Study the drawing (mm; zero at the part's minimum x, y, z) and answer. A direction names the side the tool comes from. Coordinates: 2 decimals unless noted, no trailing zeros. Order: outer loops, then holes, each group sorted by start corner. A loop starts at its lowest first (then second) coordinate and runs counter-clockwise, first axis right, second up.
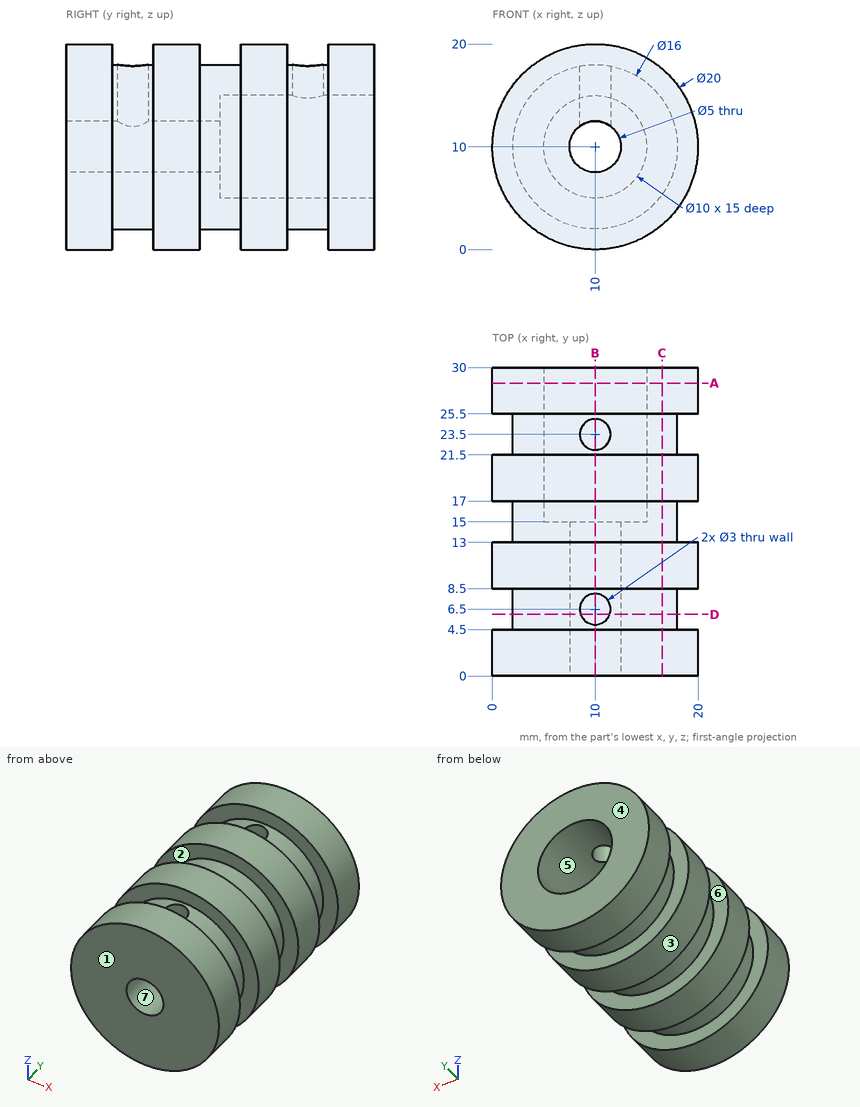
(1) Find section B-B on x = 10. Count the separate pieces of the cut face and the enclosed holes in it, then the cut area to 4 significant figures.
(2) Find section A-A on y = 28.5. Determine the outline of the cut face in (x, z).
(3) The mould has two halves that part along Y. Classify the marked faces 1, 2, 3 and 4: pulls with the +Y half, pulls with the -Y half, needs draft (parallel to the pull), parting line crosses it, or undercut.
(4) Given pin 1 Ø2 at (x, y) = (3, 17.5) entering from +Z; pin 2 Ø12 at (y, z) = (8, 17) entering from +X; pin 3 Ø1.5 at (x, y) = (11, 21) entering from +Z, each flat-ended and moving along its own axis, determine where each tip first touches the part or whether it passes through.
(5) Find section D-D on y = 6. Determine the outline of the cut face in (x, z).
(6) A tool of negligible diameter and unlimited length cuts with its end or side. For the marked faces 5, 6 and 7, from which of +Z, -Z, +X, -X, +Y, -Y can it reach the whole face along a straight path? Write none if from no direction.
(7) Find section C-C on x = 16.5. Determine the outline of the cut face in (y, z).
(8) Find the intervals of material crossed by probe 1 along Y at (x, z) = (14.75, 2.5); probe 2 along Y at (x, z) = (10, 15.5); probe 3 along X at (y, z) = (4.25, 10), in increasing order.
Resolved:
1. separate pieces: 4
1. enclosed holes: 0
1. area: 301.5 mm2
2. outline: circle Ø20 at (10, 10); hole circle Ø10 at (10, 10)
3. face 1: pulls with the -Y half
3. face 2: undercut
3. face 3: needs draft
3. face 4: pulls with the +Y half
4. pin 1: stops at z = 18
4. pin 2: stops at x = 19.95
4. pin 3: stops at z = 20
5. outline: (8.59, 12.06) - (8.59, 17.87) arc R8 ccw (long way) to (11.41, 17.87) - (11.41, 12.06) arc R2.5 cw (long way) to start
6. face 5: +Y
6. face 6: none
6. face 7: +Y, -Y
7. outline: (0, 2.4) - (4.5, 2.4) - (4.5, 5.34) - (8.5, 5.34) - (8.5, 2.4) - (13, 2.4) - (13, 5.34) - (17, 5.34) - (17, 2.4) - (21.5, 2.4) - (21.5, 5.34) - (25.5, 5.34) - (25.5, 2.4) - (30, 2.4) - (30, 17.6) - (25.5, 17.6) - (25.5, 14.66) - (21.5, 14.66) - (21.5, 17.6) - (17, 17.6) - (17, 14.66) - (13, 14.66) - (13, 17.6) - (8.5, 17.6) - (8.5, 14.66) - (4.5, 14.66) - (4.5, 17.6) - (0, 17.6) - close
8. probe 1: y = 0 to 4.5, 8.5 to 13, 17 to 21.5, 25.5 to 30
8. probe 2: y = 0 to 5, 8 to 22, 25 to 30
8. probe 3: x = 0 to 7.5, 12.5 to 20
